Could you check a few things on this drawing? It's one solid part, dimensions in mm from its lowest x, y, z. Give positions to 0.01 mm unless a question says otherwise; leave off trailing zeros. Loops run counter-clockwise (first coordinate to the right, second up) from the corner with the lowest first, then second, coordinate; pieces in that order, holes last. Notation, with made-up numbers: (-33.5, 64.5) - (-26.5, 64.5) arc R20 cw to (-26.5, 90.5) - close; hole circle Ø4 at (41, 17.5). An arc over 180 degrees is marked (long way). Answer as a JSON object with one key per item and string values.
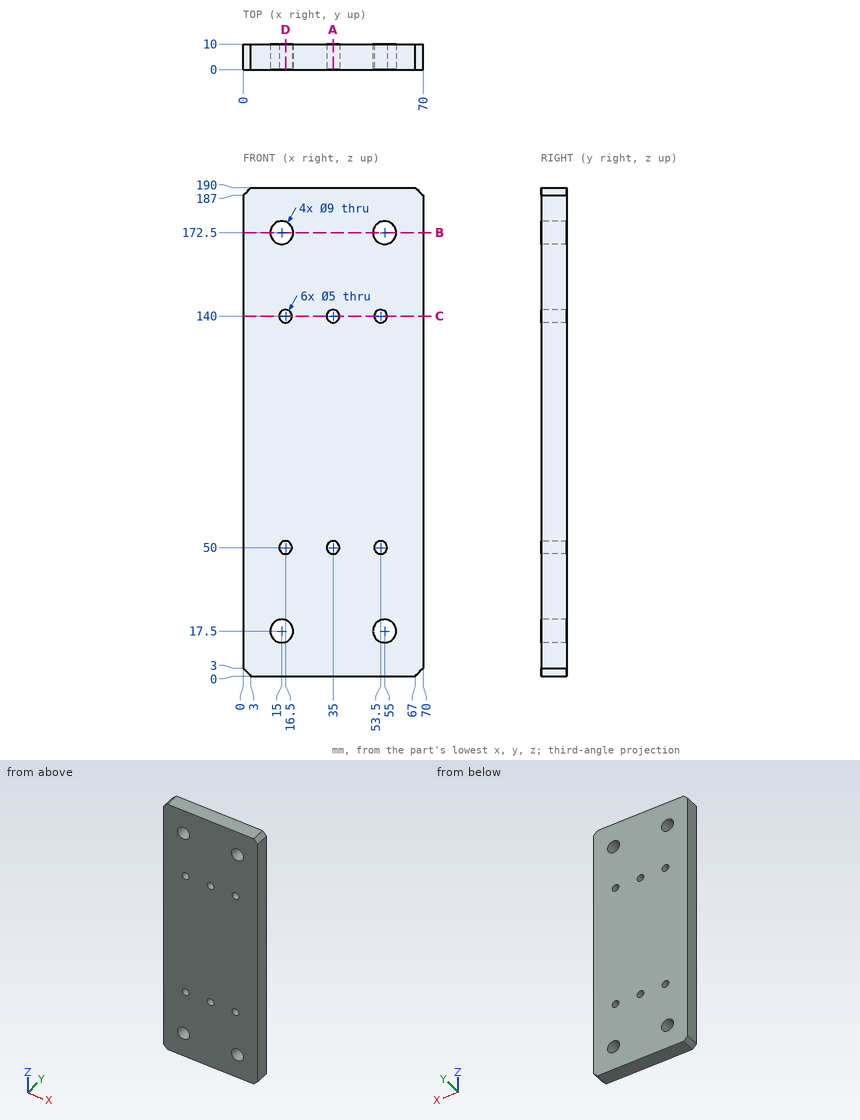
1) Imagine slicing it at D-D on x = 16.5. Write out the boundary of the cut face in (y, z), and give its area (3 significant figures).
Check sheet entries:
{"outline": "(0, 0) - (10, 0) - (10, 13.26) - (0, 13.26) - close; (0, 21.74) - (10, 21.74) - (10, 47.5) - (0, 47.5) - close; (0, 52.5) - (10, 52.5) - (10, 137.5) - (0, 137.5) - close; (0, 142.5) - (10, 142.5) - (10, 168.26) - (0, 168.26) - close; (0, 176.74) - (10, 176.74) - (10, 190) - (0, 190) - close", "area": "1,630 mm2"}
2) Imagine slicing it at C-C on z = 140. Write out the boundary of the cut face in (x, y).
Check sheet entries:
{"outline": "(0, 0) - (14, 0) - (14, 10) - (0, 10) - close; (19, 0) - (32.5, 0) - (32.5, 10) - (19, 10) - close; (37.5, 0) - (51, 0) - (51, 10) - (37.5, 10) - close; (56, 0) - (70, 0) - (70, 10) - (56, 10) - close"}
3) Imagine slicing it at A-A on x = 35. Write out the boundary of the cut face in (y, z).
Check sheet entries:
{"outline": "(0, 0) - (10, 0) - (10, 47.5) - (0, 47.5) - close; (0, 52.5) - (10, 52.5) - (10, 137.5) - (0, 137.5) - close; (0, 142.5) - (10, 142.5) - (10, 190) - (0, 190) - close"}
4) Imagine slicing it at B-B on z = 172.5. Write out the boundary of the cut face in (x, y), and give its area (3 significant figures).
Check sheet entries:
{"outline": "(0, 0) - (10.5, 0) - (10.5, 10) - (0, 10) - close; (19.5, 0) - (50.5, 0) - (50.5, 10) - (19.5, 10) - close; (59.5, 0) - (70, 0) - (70, 10) - (59.5, 10) - close", "area": "520 mm2"}
5) I need wall thicknesses on L1, parallel to X at y = 4.25, z = 17.5; L2, parallel to X at y = 6.75, z = 140; L3, parallel to Z at x = 35, y = 7.5. Which ranges of each line are inside material? Lowest first, please.
Check sheet entries:
{"L1": "0 to 10.5, 19.5 to 50.5, 59.5 to 70", "L2": "0 to 14, 19 to 32.5, 37.5 to 51, 56 to 70", "L3": "0 to 47.5, 52.5 to 137.5, 142.5 to 190"}
